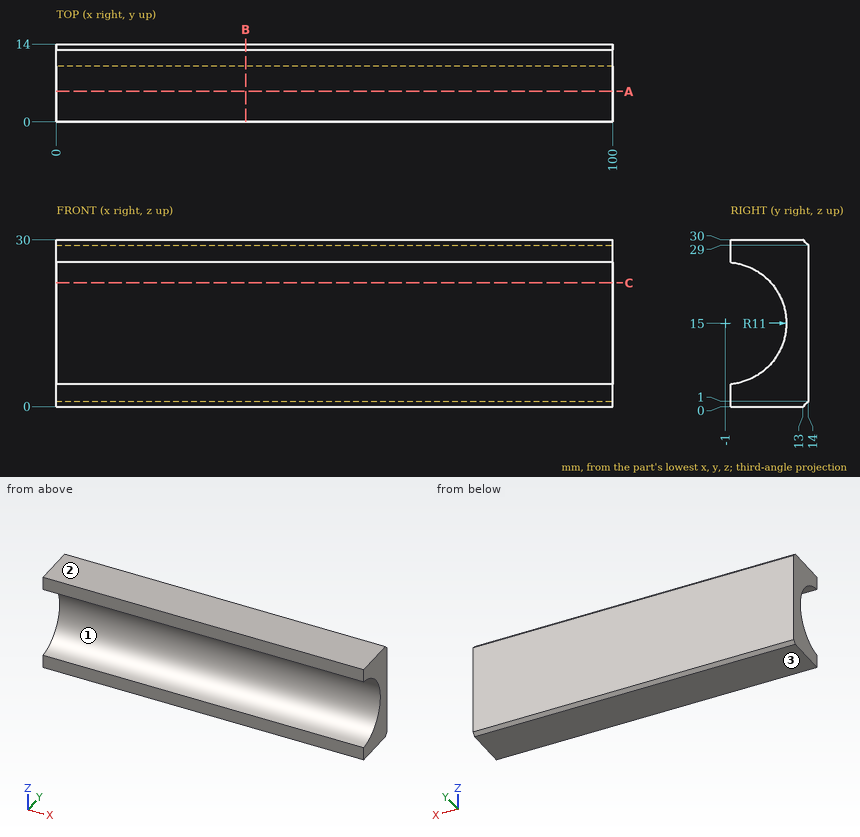
Study the drawing (mm; zero at the part's minimum x, y, z) and answer. Round coordinates to 2 decimals unless told otherwise and drop trailing zeros. Order: outer loops, then holes, each group sorted by start corner. A loop starts at its lowest first (then second) coordinate and runs counter-clockwise, first axis right, second up. Notation, with made-up numbers: (51.25, 71) -> (91.25, 71) arc R35 ccw to (91.25, 103) -> close; hole circle Ø9 at (43.5, 82). An arc over 180 degrees is marked (long way). Write each question's results on one line, items separated by ' | '. Start each with the question number.
Q1. Find section B-B (x = 34). Determine the outline of the cut face in (y, z).
Q2. This flat-tipped pin is pushed along its axis until it touches: pin 1 (8 mm diameter, centred on x = 80.5, z = 9, fed in from -Y). Where does it stop, or does it pass through?
Q3. Find section C-C (z = 22.25). Determine the outline of the cut face in (x, y), then the cut area to 3 significant figures.
Q4. Straight lines are drawn through the part: probe 1 along Z at (x, y) = (17, 2); probe 2 along Z at (x, y) = (61.5, 1); probe 3 along Y at (x, z) = (55, 15). For each, find the intervals that lie inside material, in ascending order. Write a range as from..to.
Q5. The mould has two halves that part along Z. Classify the marked faces 1, 2 and 3: pulls with the +Z half, pulls with the -Z half, needs draft (parallel to the pull), parting line crosses it, or undercut.
Q6. Find section A-A (y = 5.5). Determine the outline of the cut face in (x, z).
Worked answers:
1) outline: (0, 0) -> (13, 0) -> (14, 1) -> (14, 29) -> (13, 30) -> (0, 30) -> (0, 25.95) arc R11 cw to (0, 4.05) -> close
2) pin 1: stops at y = 3.58
3) outline: (0, 7.27) -> (100, 7.27) -> (100, 14) -> (0, 14) -> close | area: 673 mm2
4) probe 1: z = 0..4.42, 25.58..30 | probe 2: z = 0..4.18, 25.82..30 | probe 3: y = 10..14
5) face 1: undercut | face 2: pulls with the +Z half | face 3: pulls with the -Z half
6) outline: (0, 0) -> (100, 0) -> (100, 6.13) -> (0, 6.13) -> close; (0, 23.87) -> (100, 23.87) -> (100, 30) -> (0, 30) -> close
